CAD build for the part. Positions are in the model's coordinates, mm. Face numbers are marked on the shaded views. A direction names the side the tool comes from. Coordinates: 2 decimals unless noted, no trailing zeros. Loops run counter-clockwise (first coordinate to the right, second up) from the corner with the lowest first, then second, coordinate; pieces in that order, holes last.
1) Saw through at B-B, the plane z = 1.5. Write the cut outline in (x, y), and give its area (3 significant figures).
2) Which spindle directions (+Z, -Z, +X, -X, +Y, -Y) get a long thin tool onto all of the face, cutting with end or side? Do the marked faces 1 and 2. Say none if no direction does.
3) Two-plate mould, pull along Y, no slides. Class the marked faces 3, 4, 5 and 6: +Y half, -Y half, draft (parallel to the pull), parting line (faces both ways), or undercut.
4) Wall check: line 1 along Y through (x, z) = (0.25, 2.5); line 2 along Y through (x, z) = (0, -1.3); line 3 along X through (y, z) = (74.5, -0.5). Give the ranges that are in metal, low to high.
5) Saw through at A-A, the plane x = 0. Write the cut outline in (y, z).
6) Pin check, flat tips, straight feed: pin 1 Ø2 at (x, y) = (0, 45) entering from +Z; pin 2 Ø1.8 at (x, y) = (-1, 15.5) entering from -Z. Stop position of each tip, or through.
7) Saw through at C-C, the plane y = 15. Write the cut outline in (x, z), and give its area (3 significant figures).
```python
from build123d import *

# Parameters (mm, degrees)
SKETCH1_W           = 18
SKETCH1_H           = 7.5
BOSS_EXTRUDE1_DEPTH = 90
CHAMFER1_SIZE       = 1
SKETCH2_R           = 1.75
CUT_EXTRUDE1_DEPTH  = 91.759297044
SKETCH3_R           = 3
CUT_EXTRUDE2_DEPTH  = 4.5
LPATTERN1_COUNT     = 4
LPATTERN1_PITCH     = 30
LPATTERN2_COUNT     = 4
LPATTERN2_PITCH     = 30


with BuildPart() as part:
    # Sketch1 → Boss-Extrude1 (new body)
    with BuildSketch(Plane(origin=(0, 0, 0), x_dir=(1, 0, 0), z_dir=(0, 1, 0))):
        Rectangle(SKETCH1_W, SKETCH1_H)
    extrude(amount=BOSS_EXTRUDE1_DEPTH)

    # Chamfer1
    chamfer1_edges = [part.edges().sort_by_distance(p)[0] for p in [
        (-9, 45, -3.75),
        (9, 45, -3.75),
    ]]
    chamfer(chamfer1_edges, length=CHAMFER1_SIZE)

    # Sketch2 → Cut-Extrude1 (cut, through all)
    with BuildSketch(Plane(origin=(0, 0, -3.75), x_dir=(-1, 0, 0), z_dir=(0, 0, -1))):
        with Locations((0, 15)):
            Circle(SKETCH2_R)
    cut_extrude1 = extrude(amount=-CUT_EXTRUDE1_DEPTH, mode=Mode.SUBTRACT)

    # Sketch3 → Cut-Extrude2 (cut)
    with BuildSketch(Plane(origin=(0, 0, -3.75), x_dir=(-1, 0, 0), z_dir=(0, 0, -1))):
        with Locations((0, 15)):
            Circle(SKETCH3_R)
    cut_extrude2 = extrude(amount=-CUT_EXTRUDE2_DEPTH, mode=Mode.SUBTRACT)

    # LPattern1: Cut-Extrude2 ×4
    with Locations(*[(0, i * LPATTERN1_PITCH, 0) for i in range(1, LPATTERN1_COUNT)]):
        add(cut_extrude2, mode=Mode.SUBTRACT)

    # LPattern2: Cut-Extrude1 ×4
    with Locations(*[(0, i * LPATTERN2_PITCH, 0) for i in range(1, LPATTERN2_COUNT)]):
        add(cut_extrude1, mode=Mode.SUBTRACT)


solid = part.part
```
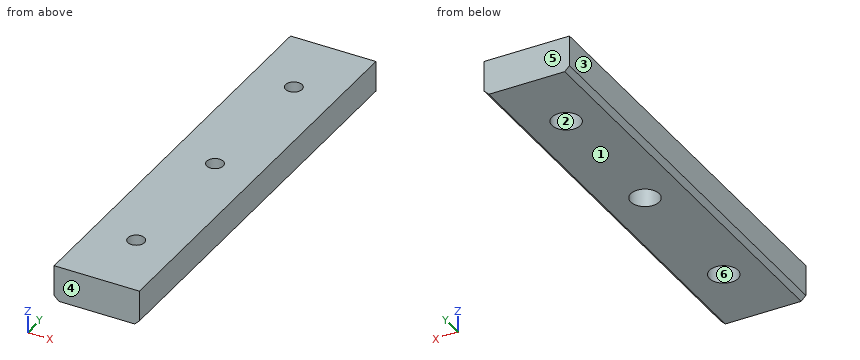
Data:
1. outline: (-9, 0) - (9, 0) - (9, 90) - (-9, 90) - close; hole circle Ø3.5 at (0, 15); hole circle Ø3.5 at (0, 45); hole circle Ø3.5 at (0, 75)
1. area: 1,590 mm2
2. face 1: -Z, +X, -X, +Y, -Y
2. face 2: -Z
3. face 3: draft
3. face 4: -Y half
3. face 5: +Y half
3. face 6: undercut
4. line 1: y = 0 to 13.27, 16.73 to 43.27, 46.73 to 73.27, 76.73 to 90
4. line 2: y = 0 to 12, 18 to 42, 48 to 72, 78 to 90
4. line 3: x = -9 to -2.96, 2.96 to 9
5. outline: (0, -3.75) - (12, -3.75) - (12, 0.75) - (13.25, 0.75) - (13.25, 3.75) - (0, 3.75) - close; (16.75, 0.75) - (18, 0.75) - (18, -3.75) - (42, -3.75) - (42, 0.75) - (43.25, 0.75) - (43.25, 3.75) - (16.75, 3.75) - close; (46.75, 0.75) - (48, 0.75) - (48, -3.75) - (72, -3.75) - (72, 0.75) - (73.25, 0.75) - (73.25, 3.75) - (46.75, 3.75) - close; (76.75, 0.75) - (78, 0.75) - (78, -3.75) - (90, -3.75) - (90, 3.75) - (76.75, 3.75) - close
6. pin 1: passes through
6. pin 2: stops at z = 0.75
7. outline: (-9, -2.75) - (-8, -3.75) - (-3, -3.75) - (-3, 0.75) - (-1.75, 0.75) - (-1.75, 3.75) - (-9, 3.75) - close; (1.75, 0.75) - (3, 0.75) - (3, -3.75) - (8, -3.75) - (9, -2.75) - (9, 3.75) - (1.75, 3.75) - close
7. area: 96.5 mm2
